Model file for the job. Use its own axes, mm. A direction names the side the tool comes from. Coordinates: 2 decimals unless noted, no trailing zeros. Order: outer loops, then holes, each group sorted by start corner. A loop starts at its lowest first (then second) coordinate and runs counter-clockwise, first axis right, second up.
from build123d import *

# Parameters (mm, degrees)
BASE_PLATE_20MM_DEPTH          = 20
MOUNTING_BOSS_RINGS_SKETCH_R   = 30
MOUNTING_BOSS_RINGS_SKETCH_R_2 = 20
MOUNTING_BOSSES_4X_60_DEPTH    = 5
TOP_NOTCH_SKETCH_R             = 20
TOP_NOTCH_CUT_DEPTH            = 397.484552032


with BuildPart() as part:
    # Plate Profile Sketch → Base Plate 20mm (new body)
    with BuildSketch(Plane.XY):
        with BuildLine():
            Line((40, 0), (90, 0))
            Line((90, 0), (90, 10))
            Line((90, 10), (130, 10))
            Line((130, 10), (130, 32.679491924))
            ThreePointArc((130, 32.679491924), (140, 70), (150, 32.679491924))
            Line((150, 32.679491924), (150, 10))
            Line((150, 10), (190, 10))
            Line((190, 10), (190, 0))
            Line((190, 0), (240, 0))
            ThreePointArc((240, 0), (268.284271247, 11.715728753), (280, 40))
            Line((280, 40), (280, 86))
            ThreePointArc((280, 86), (226, 140), (280, 194))
            Line((280, 194), (280, 240))
            ThreePointArc((280, 240), (268.284271247, 268.284271247), (240, 280))
            Line((240, 280), (190, 280))
            Line((190, 280), (190, 270))
            Line((190, 270), (150, 270))
            Line((150, 270), (150, 247.320508076))
            ThreePointArc((150, 247.320508076), (140, 210), (130, 247.320508076))
            Line((130, 247.320508076), (130, 270))
            Line((130, 270), (90, 270))
            Line((90, 270), (90, 280))
            Line((90, 280), (40, 280))
            ThreePointArc((40, 280), (11.715728753, 268.284271247), (0, 240))
            Line((0, 240), (0, 194))
            ThreePointArc((0, 194), (54, 140), (0, 86))
            Line((0, 86), (0, 40))
            ThreePointArc((0, 40), (11.715728753, 11.715728753), (40, 0))
        make_face()
    extrude(amount=BASE_PLATE_20MM_DEPTH)

    # Mounting Boss Rings Sketch → Mounting Bosses 4xØ60 (add)
    # profile 1 of 4: a face of its own
    with BuildSketch(Plane.XY.offset(20)):
        with Locations((240, 240)):
            Circle(MOUNTING_BOSS_RINGS_SKETCH_R)
        with Locations((240, 240)):
            Circle(MOUNTING_BOSS_RINGS_SKETCH_R_2, mode=Mode.SUBTRACT)
    # profile 2 of 4: a face of its own
    with BuildSketch(Plane.XY.offset(20)):
        with Locations((40, 240)):
            Circle(MOUNTING_BOSS_RINGS_SKETCH_R)
        with Locations((40, 240)):
            Circle(MOUNTING_BOSS_RINGS_SKETCH_R_2, mode=Mode.SUBTRACT)
    # profile 3 of 4: a face of its own
    with BuildSketch(Plane.XY.offset(20)):
        with Locations((240, 40)):
            Circle(MOUNTING_BOSS_RINGS_SKETCH_R)
        with Locations((240, 40)):
            Circle(MOUNTING_BOSS_RINGS_SKETCH_R_2, mode=Mode.SUBTRACT)
    # profile 4 of 4: a face of its own
    with BuildSketch(Plane.XY.offset(20)):
        with Locations((40, 40)):
            Circle(MOUNTING_BOSS_RINGS_SKETCH_R)
        with Locations((40, 40)):
            Circle(MOUNTING_BOSS_RINGS_SKETCH_R_2, mode=Mode.SUBTRACT)
    extrude(amount=MOUNTING_BOSSES_4X_60_DEPTH)

    # Top Notch Sketch → Top Notch Cut (cut, through all)
    with BuildSketch(Plane.XY.offset(20)):
        with Locations((40, 240)):
            Circle(TOP_NOTCH_SKETCH_R)
        with Locations((240, 240)):
            Circle(TOP_NOTCH_SKETCH_R)
        with Locations((240, 40)):
            Circle(TOP_NOTCH_SKETCH_R)
        with Locations((40, 40)):
            Circle(TOP_NOTCH_SKETCH_R)
    extrude(amount=-TOP_NOTCH_CUT_DEPTH, mode=Mode.SUBTRACT)


solid = part.part
Q1. Drop flat-ended pins along their axis: P1, Ø11, axis at y = 274.5, z = 6.5, coming from the +X side; P2, Ø1, axis at y = 135.5, z = 6.5, coming from the -X side; P3, Ø10, axis at x = 166.5, z = 7.5, coming from the +Y side. Give the stop position or say it passes through.
Established:
P1: stops at x = 267.55
P2: stops at x = 53.77
P3: stops at y = 270
Q2. Which spindle directions (+Z, -Z, +X, -X, +Y, -Y) get a long thin tool onto all of the face, cutting with end or side? Do faces 1 (the face through (190, 5, 10)), 2 (the face through (36.095, 269.745, 22.465)), 3 (the face through (130, 259, 10)), 4 (the face through (260, 234, 25)). Say none if no direction does.
Established:
face 1: +Z, -Z, -Y
face 2: +Z
face 3: +Z, -Z, +Y
face 4: +Z, +X, -X, +Y, -Y
Q3. Probe line 1 (Y direction, x = 234, z = 8); line 2 (Y direction, x = 240, z = 4.5); line 3 (X direction, y = 50, z = 8). List the from-to ranges inside material, lowest first.
Established:
line 1: y = 0 to 20.92, 59.08 to 111.72, 168.28 to 220.92, 259.08 to 280
line 2: y = 0 to 20, 60 to 103.72, 176.28 to 220, 260 to 280
line 3: x = 0 to 22.68, 57.32 to 120, 160 to 222.68, 257.32 to 280
Q4. Cut at C-C, the plane x = 140. List the corners of the cut face in (y, z).
Established:
outline: (70, 0) - (210, 0) - (210, 20) - (70, 20) - close
Q5. Cut at B-B, the plane y = 50. List the corners of the cut face in (x, z), plus the area to 3 significant figures.
Established:
outline: (0, 0) - (22.68, 0) - (22.68, 25) - (11.72, 25) - (11.72, 20) - (0, 20) - close; (57.32, 0) - (120, 0) - (120, 20) - (68.28, 20) - (68.28, 25) - (57.32, 25) - close; (160, 0) - (222.68, 0) - (222.68, 25) - (211.72, 25) - (211.72, 20) - (160, 20) - close; (257.32, 0) - (280, 0) - (280, 20) - (268.28, 20) - (268.28, 25) - (257.32, 25) - close
area: 3,630 mm2
Q6. Cut at D-D, the plane y = 140. List the corners of the cut face in (x, z).
Established:
outline: (54, 0) - (226, 0) - (226, 20) - (54, 20) - close
Q7. Mould opens along X. For faces 5 (the face through (190, 275, 10)), 6 (the face through (60, 234, 25)), 7 (the face through (150, 259, 10)), 8 (the face through (0, 63, 10)) say: pulls with the +X half, pulls with the -X half, needs draft (parallel to the pull), parting line crosses it, or undercut.
Established:
face 5: undercut
face 6: needs draft
face 7: undercut
face 8: pulls with the -X half
Q8. Cut at A-A, the plane z = 10.75. Count the separate pieces of the cut face and the enclosed holes in it, plus the area to 3 significant figures.
Established:
separate pieces: 1
enclosed holes: 4
area: 57,500 mm2
